For this review, take the finished solid that the model builds, in its own axes (mm). Face numbers are marked on the shaded views. A direction names the side the tool comes from. Coordinates: 2 decimals unless noted, no trailing zeros. Write each loop counter-clockwise with the first axis right and the second up, starting at its lowest first coordinate (ties: lowest second). Pieces come first, ordered by that corner, then holes.
1) To check wall thickness, follow line 1 along X through (y, z) = (-1.5, -5.75). State the ranges of the line that lie inside material, in increasing order.
2) For the marked faces 1 and 2, list the 3-axis set-ups (+Z, -Z, +X, -X, +Y, -Y) from which the entire face can be reached by the end or side of a thin tool; tool diameter is ignored.
3) We need section A-A on z = 0. Write out the cut boundary in (x, y), then the cut area to 3 significant figures.
4) We need section D-D on x = -6. Write out the cut boundary in (y, z), then the cut area to 3 significant figures.
5) Insertion check: P1, Ø1.5, axis at y = 4, z = -3.5, coming from the -X side; P2, Ø4, axis at x = 23.5, y = 0.5, coming from the -Z side; P3, Ø2, axis at x = 1.5, z = 4.5, coming from the -Y side; P4, Ø4, axis at x = 18, y = -3.5, coming from the -Z side. Each pin has a flat end and moves straight along its axis. Give the tip position at first contact, or say it passes through.
6) We need section C-C on x = -20. Write out the cut boundary in (y, z), then the cut area to 3 significant figures.
from build123d import *

# Parameters (mm, degrees)
SKETCH2_W = 1
SKETCH2_H = 2.2


with BuildPart() as part:
    # Sketch1 → Revolve1 (revolve)
    with BuildSketch(Plane.XY, mode=Mode.PRIVATE) as revolve1_sk:
        Polygon((-11, 0), (-11, 3), (36, 3), (36, 8), (38.5, 8), (38.5, 0), align=None)
    revolve(revolve1_sk.sketch.rotate(Axis((38.5, 0, 0), (-1, 0, 0)), 90), axis=Axis((38.5, 0, 0), (-1, 0, 0)))

    # Sketch2 → Revolve2 (revolve)
    with BuildSketch(Plane.XY, mode=Mode.PRIVATE) as revolve2_sk:
        with Locations((-11.5, 1.1)):
            Rectangle(SKETCH2_W, SKETCH2_H)
    revolve(revolve2_sk.sketch.rotate(Axis((-11, 0, 0), (-1, 0, 0)), 90), axis=Axis((-11, 0, 0), (-1, 0, 0)))

    # Sketch3 → Revolve3 (revolve)
    with BuildSketch(Plane.XY, mode=Mode.PRIVATE) as revolve3_sk:
        Polygon((-24, 0), (-24, 2.0095), (-23.5095, 2.5), (-12, 2.5), (-12, 0), align=None)
    revolve(revolve3_sk.sketch.rotate(Axis((-12, 0, 0), (-1, 0, 0)), 90), axis=Axis((-12, 0, 0), (-1, 0, 0)))


solid = part.part
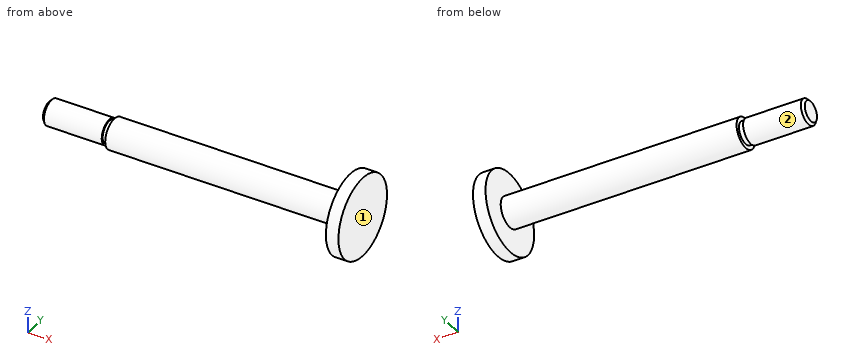
Result:
1. line 1: x = 36 to 38.5
2. face 1: +Z, -Z, +X, +Y, -Y
2. face 2: -X
3. outline: (-24, -2.01) - (-23.51, -2.5) - (-12, -2.5) - (-12, -2.2) - (-11, -2.2) - (-11, -3) - (36, -3) - (36, -8) - (38.5, -8) - (38.5, 8) - (36, 8) - (36, 3) - (-11, 3) - (-11, 2.2) - (-12, 2.2) - (-12, 2.5) - (-23.51, 2.5) - (-24, 2.01) - close
3. area: 386 mm2
4. outline: circle Ø6 at (0, 0)
4. area: 28.3 mm2
5. P1: stops at x = 36
5. P2: stops at z = -3
5. P3: passes through
5. P4: stops at z = -2.6
6. outline: circle Ø5 at (0, 0)
6. area: 19.6 mm2
